For this review, use the dimensioned drawing (mm, ordinates from the lowest corner) and the shaded views. A direction names the side the tool comes from. Round coordinates to 2 decimals unless told otherwise and drop trailing zeros. Write each loop counter-clockwise with the first axis right and the second up, starting at its lowest first coordinate (ties: lowest second). Pieces come first, ordered by that corner, then holes.
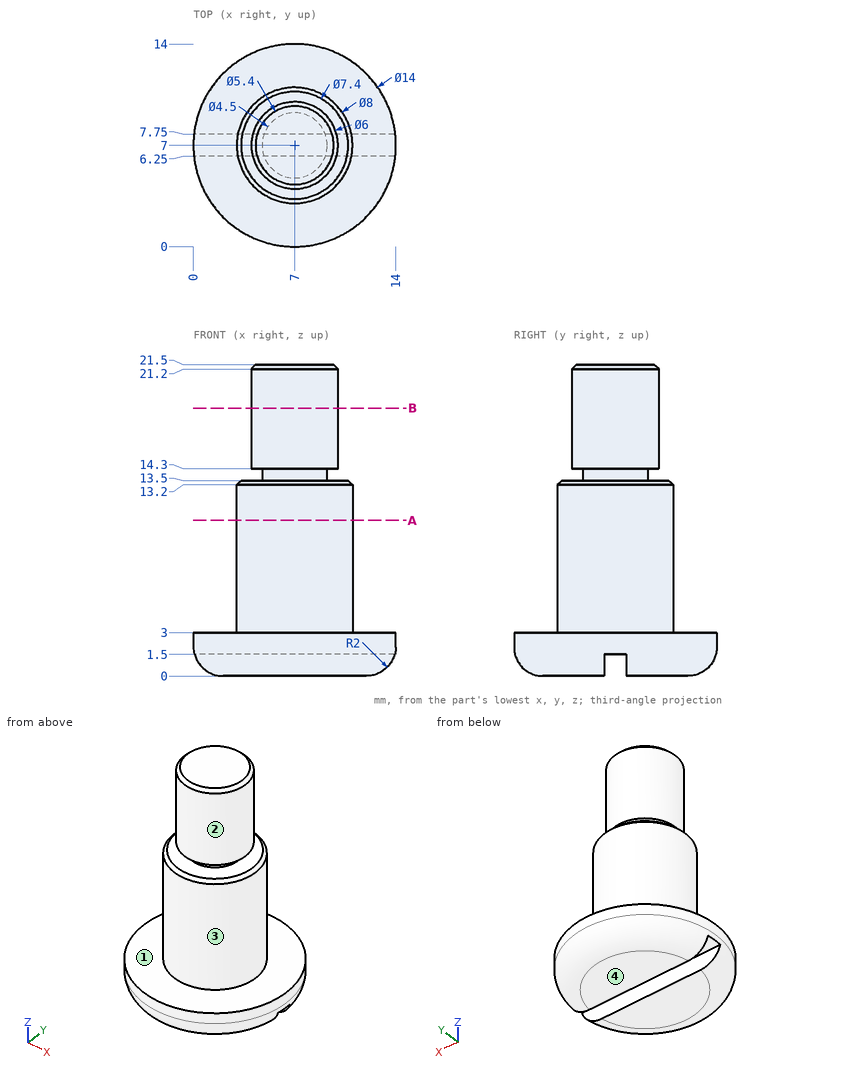
(1) For line 1 along Z through (x, y) = (6.5, 11); line 2 along Y through (x, z) = (7, 7.5); line 3 along Z through (x, y) = (1.5, 7.25), list the stretches that pass through material, from the lowest coordinate up.
Geometry check:
line 1: z = 0 to 3
line 2: y = 3 to 11
line 3: z = 1.5 to 3
(2) We need section A-A, the plane z = 10.75. Give the boundary of the cut face in (x, y).
Geometry check:
outline: circle Ø8 at (7, 7)
(3) For the marked faces 3 and 4, list the 3-axis set-ups (+Z, -Z, +X, -X, +Y, -Y) from which the entire face can be reached by the end or side of a thin tool; tool diameter is ignored.
Geometry check:
face 3: +Z
face 4: -Z, +X, -X, +Y, -Y
(4) We need section B-B, the plane z = 18.5. Give the boundary of the cut face in (x, y), and give its area (3 significant figures).
Geometry check:
outline: circle Ø6 at (7, 7)
area: 28.3 mm2
(5) Mouldability with a two-part tool opening along X and no side actions: class the marked faces 1 and 2 as pulls with the +X half, pulls with the -X half, needs draft (parallel to the pull), parting line crosses it, or undercut.
Geometry check:
face 1: needs draft
face 2: parting line crosses it
(6) For pin 1 Ø1 at (x, z) = (11, 19) entering from -Y; pin 2 Ø6 at (x, z) = (2.5, 14.5) entering from -Y; pin 3 Ø1.5 at (x, z) = (3, 2.5) entering from +Y; pin 4 Ø3 at (x, y) = (2, 11.5) entering from -Z, all flat-tipped, find the tip position at first contact; note any pin that passes through.
Geometry check:
pin 1: passes through
pin 2: stops at y = 3.43
pin 3: stops at y = 13.2
pin 4: stops at z = 0.01
